Could you check a few things on this model? Use its own coordinates, in mm. Coordinates: 2 decimals unless noted, no trailing zeros. Loops run counter-clockwise (first coordinate to the right, second up) from the corner with the lowest first, then second, coordinate; pieces in that order, holes last.
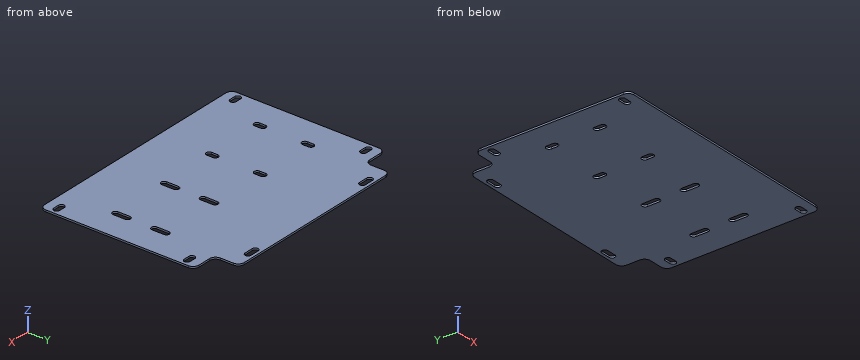
from build123d import *

# Parameters (mm, degrees)
SKETCH1_W           = 400
SKETCH1_H           = 342
BOSS_EXTRUDE1_DEPTH = 3
SKETCH3_W           = 86.448848967
SKETCH3_H           = 526.142419803
CUT_EXTRUDE2_DEPTH  = 527.282243668
FILLET1_R           = 10
CUT_EXTRUDE3_DEPTH  = 527.282243668
SKETCH5_W           = 336
SKETCH5_H           = 215.570811559
CUT_EXTRUDE4_DEPTH  = 10


with BuildPart() as part:
    # Sketch1 → Boss-Extrude1 (new body)
    with BuildSketch(Plane.XY):
        with Locations((200, -171)):
            Rectangle(SKETCH1_W, SKETCH1_H)
        with BuildLine():
            Line((253, -128.5), (253, -148.5))
            ThreePointArc((253, -148.5), (248, -153.5), (243, -148.5))
            Line((243, -148.5), (243, -128.5))
            ThreePointArc((243, -128.5), (248, -123.5), (253, -128.5))
        make_face(mode=Mode.SUBTRACT)
        with BuildLine():
            Line((345, -128.5), (345, -148.5))
            ThreePointArc((345, -148.5), (350, -153.5), (355, -148.5))
            Line((355, -148.5), (355, -128.5))
            ThreePointArc((355, -128.5), (350, -123.5), (345, -128.5))
        make_face(mode=Mode.SUBTRACT)
        with BuildLine():
            Line((345, -213.5), (345, -193.5))
            ThreePointArc((345, -193.5), (350, -188.5), (355, -193.5))
            Line((355, -193.5), (355, -213.5))
            ThreePointArc((355, -213.5), (350, -218.5), (345, -213.5))
        make_face(mode=Mode.SUBTRACT)
        with BuildLine():
            Line((253, -213.5), (253, -193.5))
            ThreePointArc((253, -193.5), (248, -188.5), (243, -193.5))
            Line((243, -193.5), (243, -213.5))
            ThreePointArc((243, -213.5), (248, -218.5), (253, -213.5))
        make_face(mode=Mode.SUBTRACT)
        with BuildLine():
            Line((72.5, -5), (87.5, -5))
            ThreePointArc((87.5, -5), (92.5, -10), (87.5, -15))
            Line((87.5, -15), (72.5, -15))
            ThreePointArc((72.5, -15), (67.5, -10), (72.5, -5))
        make_face(mode=Mode.SUBTRACT)
        with BuildLine():
            Line((327.5, -5), (312.5, -5))
            ThreePointArc((312.5, -5), (307.5, -10), (312.5, -15))
            Line((312.5, -15), (327.5, -15))
            ThreePointArc((327.5, -15), (332.5, -10), (327.5, -5))
        make_face(mode=Mode.SUBTRACT)
        with BuildLine():
            Line((327.5, -337), (312.5, -337))
            ThreePointArc((312.5, -337), (307.5, -332), (312.5, -327))
            Line((312.5, -327), (327.5, -327))
            ThreePointArc((327.5, -327), (332.5, -332), (327.5, -337))
        make_face(mode=Mode.SUBTRACT)
        with BuildLine():
            Line((72.5, -337), (87.5, -337))
            ThreePointArc((87.5, -337), (92.5, -332), (87.5, -327))
            Line((87.5, -327), (72.5, -327))
            ThreePointArc((72.5, -327), (67.5, -332), (72.5, -337))
        make_face(mode=Mode.SUBTRACT)
        with BuildLine():
            Line((55, -126), (55, -136))
            ThreePointArc((55, -136), (50, -141), (45, -136))
            Line((45, -136), (45, -126))
            ThreePointArc((45, -126), (50, -121), (55, -126))
        make_face(mode=Mode.SUBTRACT)
        with BuildLine():
            Line((155, -126), (155, -136))
            ThreePointArc((155, -136), (150, -141), (145, -136))
            Line((145, -136), (145, -126))
            ThreePointArc((145, -126), (150, -121), (155, -126))
        make_face(mode=Mode.SUBTRACT)
        with BuildLine():
            Line((155, -216), (155, -206))
            ThreePointArc((155, -206), (150, -201), (145, -206))
            Line((145, -206), (145, -216))
            ThreePointArc((145, -216), (150, -221), (155, -216))
        make_face(mode=Mode.SUBTRACT)
        with BuildLine():
            Line((55, -216), (55, -206))
            ThreePointArc((55, -206), (50, -201), (45, -206))
            Line((45, -206), (45, -216))
            ThreePointArc((45, -216), (50, -221), (55, -216))
        make_face(mode=Mode.SUBTRACT)
    extrude(amount=BOSS_EXTRUDE1_DEPTH)

    # Sketch3 → Cut-Extrude2 (cut, through all)
    with BuildSketch(Plane.XY.offset(3)):
        with Locations((-1.224424484, -563.071209901)):
            Rectangle(SKETCH3_W, SKETCH3_H)
        with Locations((401.224424484, -563.071209901)):
            Rectangle(SKETCH3_W, SKETCH3_H)
        with Locations((401.224424484, 221.071209902)):
            Rectangle(SKETCH3_W, SKETCH3_H)
        with Locations((-1.224424484, 221.071209902)):
            Rectangle(SKETCH3_W, SKETCH3_H)
    extrude(amount=-CUT_EXTRUDE2_DEPTH, mode=Mode.SUBTRACT)

    # Fillet1
    fillet1_edges = [part.edges().sort_by_distance(p)[0] for p in [
        (358, 0, 1.5),
        (42, 0, 1.5),
        (400, -300, 1.5),
        (400, -42, 1.5),
        (42, -342, 1.5),
        (358, -342, 1.5),
        (0, -300, 1.5),
        (0, -42, 1.5),
        (42, -42, 1.5),
        (358, -42, 1.5),
        (358, -300, 1.5),
        (42, -300, 1.5),
    ]]
    fillet(fillet1_edges, radius=FILLET1_R)

    # Sketch4 → Cut-Extrude3 (cut, through all)
    with BuildSketch(Plane.XY.offset(3)):
        with BuildLine():
            Line((10, -57), (20, -57))
            ThreePointArc((20, -57), (25, -62), (20, -67))
            Line((20, -67), (10, -67))
            ThreePointArc((10, -67), (5, -62), (10, -57))
        make_face()
        with BuildLine():
            Line((390, -57), (380, -57))
            ThreePointArc((380, -57), (375, -62), (380, -67))
            Line((380, -67), (390, -67))
            ThreePointArc((390, -67), (395, -62), (390, -57))
        make_face()
        with BuildLine():
            Line((390, -285), (380, -285))
            ThreePointArc((380, -285), (375, -280), (380, -275))
            Line((380, -275), (390, -275))
            ThreePointArc((390, -275), (395, -280), (390, -285))
        make_face()
        with BuildLine():
            Line((10, -285), (20, -285))
            ThreePointArc((20, -285), (25, -280), (20, -275))
            Line((20, -275), (10, -275))
            ThreePointArc((10, -275), (5, -280), (10, -285))
        make_face()
    extrude(amount=-CUT_EXTRUDE3_DEPTH, mode=Mode.SUBTRACT)

    # Sketch5 → Cut-Extrude4 (cut)
    with BuildSketch(Plane.XY.offset(3)):
        with Locations((200, -407.78540578)):
            Rectangle(SKETCH5_W, SKETCH5_H)
    extrude(amount=-CUT_EXTRUDE4_DEPTH, mode=Mode.SUBTRACT)


solid = part.part
(1) I need wall thicknesses on probe 1 along X at (y, z) = (-132.5, 1.95); probe 2 along Y at (x, z) = (80.5, 0.4); probe 3 along Y at (x, z) = (247, 2.75). Which ranges of each line are inside material? Lowest first, please.
Answers:
probe 1: x = 0 to 45, 55 to 145, 155 to 243, 253 to 345, 355 to 400
probe 2: y = -300 to -15, -5 to 0
probe 3: y = -300 to -218.4, -188.6 to -153.4, -123.6 to 0
(2) For pin 1 (1.5 mm diameter, centred on y = -33, z = 0.5, fed in from +X); pin 2 (1.5 mm diameter, centred on y = -33.5, z = 1, fed in from +X); pin 3 (1.5 mm diameter, centred on x = 12.5, z = 1, fed in from +Y), each with a flat end and sliding along its axis, tell me the tip position at first contact or that it passes through.
Answers:
pin 1: stops at x = 358.15
pin 2: stops at x = 358.26
pin 3: stops at y = -42
(3) Imagine slicing it at B-B, the plane z = 1. State how many separate pieces and enclosed holes the cut face has, and give its area (3 significant figures).
Answers:
separate pieces: 1
enclosed holes: 14
area: 113,000 mm2
(4) Imagine slicing it at A-A, the plane y = -280. Write out the boundary of the cut face in (x, z).
Answers:
outline: (0, 0) - (5, 0) - (5, 3) - (0, 3) - close; (25, 0) - (375, 0) - (375, 3) - (25, 3) - close; (395, 0) - (400, 0) - (400, 3) - (395, 3) - close
(5) Imagine slicing it at C-C, the plane x = 37. Write out the boundary of the cut face in (y, z), and give its area (3 significant figures).
Answers:
outline: (-300, 0) - (-40.66, 0) - (-40.66, 3) - (-300, 3) - close
area: 778 mm2
